Input: part model. Units: mm. Frame: model coordinates. Face numbers are marked on the shaded views. A direction names the side the tool comes from. Give positions to 0.01 mm unless a question says otherwise; leave off trailing zeros. Write each loop counter-clockwise with the first axis right and the second up, starting at its lowest first coordinate (ties: lowest second). Pieces come first, ordered by that corner, then holes. Notation, with made-up numbers: (-16.75, 27.25) - (1.25, 27.25) arc R29 ccw to (1.25, 65.25) - close; hole circle Ø6 at (-21, 81). An arc over 180 degrees is marked (long way). Use a Markdown table: item, result. Add a question column.
1. Material intervals for probe 1 along Y at (x, z) = (0, -4.1); probe 2 along Y at (x, z) = (0, 3.6); probe 3 along Z at (x, y) = (-3.25, -8.75), sorted ascending.
2. Section query A-A, the plane z = 1.25. Return loops of the section in (x, y).
3. Set-up query: the marked faces 1, 2 and 3. Return all of +Z, -Z, +X, -X, +Y, -Y with unobstructed straight access to the full face (end or side cutting, diameter ignored); none if empty.
4. Pin query (flat end, axial travel): pin 1 (1 mm diameter, centred on y = -6, z = 1, fed in from +X) (3 decimals); pin 2 (2 mm diameter, centred on x = 7.5, z = -1, fed in from -Y); pin 3 (1 mm diameter, centred on x = 1.5, z = -2, fed in from -Y); pin 4 (11.5 mm diameter, centred on x = 0, y = 0, fed in from +Z). Return the tip coordinate at first contact, or that it passes through.
5. Mould query, pull axis X, two halves, no side actions, for the marked faces 4, 5 and 6. Classes: released by +X, released by -X, zero draft, split by the parting line, or undercut.
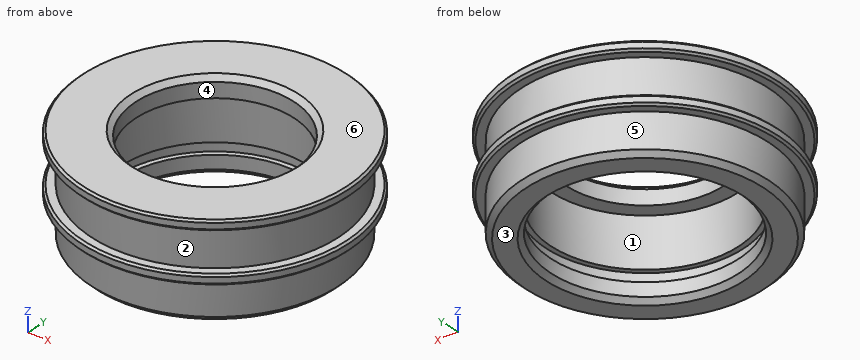
```python
from build123d import *

# Parameters (mm, degrees)
SKETCH_1_R          = 12.5
SKETCH_1_R_2        = 8
EXTRUDE_1_DEPTH     = 4
SKETCH_2_R          = 13.5
SKETCH_2_R_2        = 8
EXTRUDE_2_DEPTH     = 1
EXTRUDE_START       = 1
SKETCH_3_R          = 13.5
SKETCH_3_R_2        = 8
EXTRUDE_3_DEPTH     = 1
SKETCH_4_R          = 9.5
CUT_EXTRUDE_1_DEPTH = 4
EXTRUDE_START_2     = 4
SKETCH_7_R          = 12.5
SKETCH_7_R_2        = 9.5
EXTRUDE_4_DEPTH     = 4
CUT_EXTRUDE_START   = -3
SKETCH_8_R          = 10
SKETCH_8_R_2        = 6
CUT_EXTRUDE_2_DEPTH = 1.15
CHAMFER_1_SIZE      = 0.5
CHAMFER_2_SIZE      = 0.2


with BuildPart() as part:
    # 草图1 → 凸台-拉伸1 (new body)
    with BuildSketch(Plane.XY):
        Circle(SKETCH_1_R)
        Circle(SKETCH_1_R_2, mode=Mode.SUBTRACT)
    extrude(amount=EXTRUDE_1_DEPTH)

    # 草图2 → 凸台-拉伸2 (add)
    with BuildSketch(Plane.XY.offset(4)):
        Circle(SKETCH_2_R)
        Circle(SKETCH_2_R_2, mode=Mode.SUBTRACT)
    extrude(amount=EXTRUDE_2_DEPTH)

    # 草图3 → 凸台-拉伸3 (add)
    with BuildSketch(Plane(origin=(0, 0, 0), x_dir=(-1, 0, 0), z_dir=(0, 0, -1)).offset(EXTRUDE_START)):
        with Locations(Location((0, 0, 0), (0, 0, 180))):
            Circle(SKETCH_3_R)
        Circle(SKETCH_3_R_2, mode=Mode.SUBTRACT)
    extrude(amount=-EXTRUDE_3_DEPTH)

    # 草图4 → 切除-拉伸1 (cut)
    with BuildSketch(Plane(origin=(0, 0, -1), x_dir=(-1, 0, 0), z_dir=(0, 0, -1))):
        Circle(SKETCH_4_R)
    extrude(amount=-CUT_EXTRUDE_1_DEPTH, mode=Mode.SUBTRACT)

    # 草图7 → 凸台-拉伸4 (add)
    with BuildSketch(Plane(origin=(0, 0, -1), x_dir=(-1, 0, 0), z_dir=(0, 0, -1)).offset(EXTRUDE_START_2)):
        Circle(SKETCH_7_R)
        Circle(SKETCH_7_R_2, mode=Mode.SUBTRACT)
    extrude(amount=-EXTRUDE_4_DEPTH)

    # 草图8 → 切除-拉伸2 (cut)
    with BuildSketch(Plane(origin=(0, 0, -5), x_dir=(-1, 0, 0), z_dir=(0, 0, -1)).offset(CUT_EXTRUDE_START)):
        Circle(SKETCH_8_R)
        Circle(SKETCH_8_R_2, mode=Mode.SUBTRACT)
    extrude(amount=CUT_EXTRUDE_2_DEPTH, mode=Mode.SUBTRACT)

    # 倒角1
    chamfer_1_edges = [part.edges().sort_by_distance(p)[0] for p in [
        (-8, 0, 5),
        (12.5, 0, -5),
        (9.5, 0, -5),
    ]]
    chamfer(chamfer_1_edges, length=CHAMFER_1_SIZE)

    # 倒角2
    chamfer_2_edges = [part.edges().sort_by_distance(p)[0] for p in [
        (-13.5, 0, 4),
        (-13.5, 0, -1),
        (-13.5, 0, 0),
        (-13.5, 0, 5),
    ]]
    chamfer(chamfer_2_edges, length=CHAMFER_2_SIZE)


solid = part.part
```
Result sheet:
| question | item | result |
|---|---|---|
| 1 | probe 1 | y = -12.5 to -9.5, 9.5 to 12.5 |
| 1 | probe 2 | y = -12.5 to -8, 8 to 12.5 |
| 1 | probe 3 | z = 3 to 5 |
| 2 | outline | circle Ø25 at (0, 0); hole circle Ø19 at (0, 0) |
| 3 | face 1 | -Z |
| 3 | face 2 | none |
| 3 | face 3 | -Z, +X, -X, +Y, -Y |
| 4 | pin 1 | stops at x = 11.225 |
| 4 | pin 2 | stops at y = -11.82 |
| 4 | pin 3 | stops at y = -12.46 |
| 4 | pin 4 | passes through |
| 5 | face 4 | undercut |
| 5 | face 5 | split by the parting line |
| 5 | face 6 | zero draft |
